```python
from build123d import *

# Parameters (mm, degrees)
BASE_BLOCK_PROFILE_W   = 200
BASE_BLOCK_PROFILE_H   = 175
BASE_BLOCK_DEPTH       = 50
NOTCHED_BOSS_175_DEPTH = 175
NOTCHED_BOSS_200_DEPTH = 200


with BuildPart() as part:
    # Base Block Profile → Base Block (new body)
    with BuildSketch(Plane.XY):
        with Locations((100, 87.5)):
            Rectangle(BASE_BLOCK_PROFILE_W, BASE_BLOCK_PROFILE_H)
    extrude(amount=-BASE_BLOCK_DEPTH)

    # Notched Boss Profile 175 → Notched Boss 175 (add)
    with BuildSketch(Plane.XZ):
        Polygon((100, 75), (15, 0), (185, 0), align=None)
    extrude(amount=-NOTCHED_BOSS_175_DEPTH)

    # Notched Boss Profile 200 → Notched Boss 200 (add)
    with BuildSketch(Plane(origin=(200, 0, 0), x_dir=(0, 0, -1), z_dir=(1, 0, 0))):
        Polygon((0, 50), (0, 125), (-50, 125), (-50, 110), (-15, 110), (-15, 65), (-50, 65), (-50, 50), (-15, 50), align=None)
    extrude(amount=-NOTCHED_BOSS_200_DEPTH)


solid = part.part
```
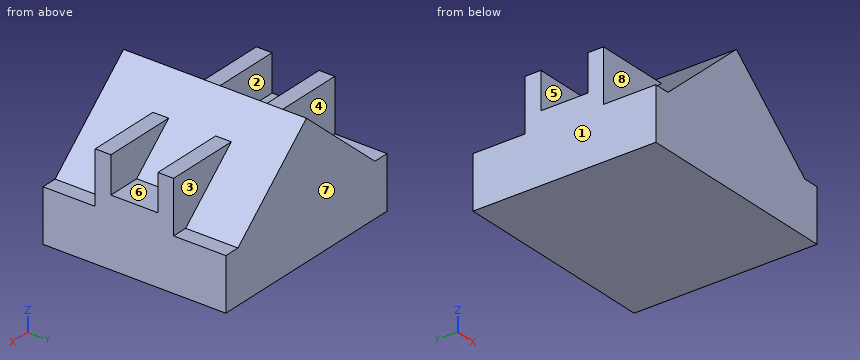
Here's how the part is built. I have some questions about the finished solid (model axes, mm). Face numbers are marked on the shaded views. A direction names the side the tool comes from. Coordinates: 2 decimals unless noted, no trailing zeros. Write each loop counter-clockwise with the first axis right and the second up, starting at its lowest first coordinate (ties: lowest second). Pieces come first, ordered by that corner, then holes. Notation, with made-up numbers: M 13.5,31.25 L 43.5,31.25 A15 cw 43.5,49.25 Z; hole C -31.5,56 d6. An arc over 180 degrees is marked long. Answer as CSV lines item,"result". Start each with the question number.
Q1. For the marked faces 4, 5, 6, 7 and 8, which set-ups out of +Z, -Z, +X, -X, +Y, -Y let a thin tool reach every point of the face, with its end or its side?
Q2. Suppose I cut it at C-C, the plane y = 79.5. List the corners of the cut face in (x, z) for me.
Q3. Will these pins go through, and if not, where does the flat tip stop? pin 1 Ø10 at (x, z) = (28, 21.5) entering from +Y; pin 2 Ø9.5 at (x, y) = (20.5, 78) entering from +Z; pin 3 Ø7.5 at (x, y) = (169.5, 59.5) entering from +Z.
Q4. Suppose I cut it at B-B, the plane x = 53.5. List the corners of the cut face in (y, z) for me.
Q5. Suppose I cut it at D-D, the plane z = 5. List the corners of the cut face in (x, y) for me.
Q6. Suppose I cut it at A-A, the plane y = 162. List the corners of the cut face in (x, z) for me.
Q7. I need wall thicknesses on probe 1 along Y at (x, z) = (17.5, 39); probe 2 along Z at (x, y) = (14, 138.5); probe 3 along Z at (x, y) = (23, 53). Which ranges of each line are inside material? Lowest first, please. Write a range as [from, to].
Q8. If we mould it in two halves opening along Y, with no side actions, what happens to the marked faces 1, 2 and 3? For each: pulls with the +Y half, pulls with the -Y half, needs draft (parallel to the pull), parting line crosses it, or undercut.
Entries:
1,face 4,"+Z, -X, +Y"
1,face 5,"+Z, -X"
1,face 6,"+Z, +X"
1,face 7,"+Z, -Z, +X, -X, +Y"
1,face 8,"+Z, -X, -Y"
2,outline,"M 0,-50 L 200,-50 L 200,15 L 168,15 L 100,75 L 32,15 L 0,15 Z"
3,pin 1,"stops at y = 125"
3,pin 2,"stops at z = 15"
3,pin 3,"stops at z = 50"
4,outline,"M 0,-50 L 175,-50 L 175,33.97 L 125,33.97 L 125,50 L 110,50 L 110,33.97 L 65,33.97 L 65,50 L 50,50 L 50,33.97 L 0,33.97 Z"
5,outline,"M 0,50 L 20.67,50 L 20.67,0 L 179.33,0 L 179.33,50 L 200,50 L 200,125 L 179.33,125 L 179.33,175 L 20.67,175 L 20.67,125 L 0,125 Z"
6,outline,"M 0,-50 L 200,-50 L 200,0 L 185,0 L 100,75 L 15,0 L 0,0 Z"
7,probe 1,"y = [50, 65], [110, 125]"
7,probe 2,"z = [-50, 0]"
7,probe 3,"z = [-50, 50]"
8,face 1,"needs draft"
8,face 2,"undercut"
8,face 3,"pulls with the +Y half"
